from build123d import *

# Parameters (mm, degrees)
BASE_BODY_PROFILE_R   = 6.5
BASE_BODY_DEPTH       = 36
POCKET_32X20_SKETCH_W = 32
POCKET_32X20_SKETCH_H = 24
POCKET_32X20_DEPTH    = 110.840793879
LUG_ROUNDED_TOP_DEPTH = 14
LUG_BORE_34_REACH     = 128.4
LUG_BORE_SKETCH_R     = 17
BOSS_10MM_DEPTH       = 10
BOSS_BORE_SKETCH_R    = 12
BOSS_BORE_24_DEPTH    = 123.036879672


with BuildPart() as part:
    # Base Body Profile → Base Body (new, symmetric)
    with BuildSketch(Plane.XY):
        with BuildLine():
            Line((0, -12), (0, 0))
            Line((0, 0), (0, 55))
            Line((0, 55), (-14, 55))
            Line((-14, 55), (-14, 30))
            Line((-14, 30), (-28, 30))
            ThreePointArc((-28, 30), (-33.656854249, 27.656854249), (-36, 22))
            Line((-36, 22), (-36, 12))
            Line((-36, 12), (-94, 12))
            Line((-94, 12), (-94, 0))
            Line((-94, 0), (-88, 0))
            Line((-88, 0), (-88, -12))
            ThreePointArc((-88, -12), (-76, -24), (-64, -12))
            Line((-64, -12), (0, -12))
        make_face()
        with Locations((-76, -12)):
            Circle(BASE_BODY_PROFILE_R, mode=Mode.SUBTRACT)
    extrude(amount=BASE_BODY_DEPTH, both=True)

    # Pocket 32x20 Sketch → Pocket 32x20 (cut, through all)
    with BuildSketch(Plane.ZY.offset(88)):
        with Locations((0, -12)):
            Rectangle(POCKET_32X20_SKETCH_W, POCKET_32X20_SKETCH_H)
    extrude(amount=-POCKET_32X20_DEPTH, mode=Mode.SUBTRACT)

    # Lug Rounded Top Sketch → Lug Rounded Top (add)
    with BuildSketch(Plane(origin=(0, 0, 0), x_dir=(0, 0, -1), z_dir=(1, 0, 0))):
        with BuildLine():
            Line((-36, 55), (36, 55))
            ThreePointArc((36, 55), (0, 91), (-36, 55))
        make_face()
    extrude(amount=-LUG_ROUNDED_TOP_DEPTH)

    # Lug Bore Sketch → Lug Bore Ø34 (cut, up to next)
    with BuildSketch(Plane.ZY.offset(14), mode=Mode.PRIVATE) as lug_bore_34_sk1:
        with Locations(Location((0, 55, 0), (0, 0, 270))):
            Circle(LUG_BORE_SKETCH_R)
    lug_bore_34_tool1 = extrude(lug_bore_34_sk1.sketch, amount=-LUG_BORE_34_REACH, mode=Mode.PRIVATE) & part.part
    add(lug_bore_34_tool1.solids().sort_by_distance((-14, 55, 0))[0], mode=Mode.SUBTRACT)

    # Boss Profile 44x30 → Boss 10mm (add)
    with BuildSketch(Plane(origin=(0, 12, 0), x_dir=(1, 0, 0), z_dir=(0, 1, 0))):
        with BuildLine():
            Line((-66, 22), (-36, 22))
            Line((-36, 22), (-36, -22))
            Line((-36, -22), (-66, -22))
            ThreePointArc((-66, -22), (-88, 0), (-66, 22))
        make_face()
    extrude(amount=BOSS_10MM_DEPTH)

    # Boss Bore Sketch → Boss Bore Ø24 (cut, through all)
    with BuildSketch(Plane(origin=(0, 22, 0), x_dir=(1, 0, 0), z_dir=(0, 1, 0))):
        with Locations(Location((-66, 0, 0), (0, 0, 180))):
            Circle(BOSS_BORE_SKETCH_R)
    extrude(amount=-BOSS_BORE_24_DEPTH, mode=Mode.SUBTRACT)


solid = part.part
Geometry: final body of the model. Coordinates: model frame, mm. A direction names the side the tool comes from. Give positions to 0.01 mm unless a question says otherwise; leave off trailing zeros. Loops run counter-clockwise (first coordinate to the right, second up) from the corner with the lowest first, then second, coordinate; pieces in that order, holes last. Notation, with made-up numbers: (55, -28) -> (75, -28) arc R21 ccw to (75, 10) -> close; hole circle Ø9 at (41, 53). An arc over 180 degrees is marked (long way). Put each result on its own line as item: value.
1. Cut plane C-C (x = -76). Return the cut outline in (y, z).
Taken from the geometry:
outline: (-24, -36) -> (-18.5, -36) -> (-18.5, -16) -> (-24, -16) -> close; (-24, 16) -> (-18.5, 16) -> (-18.5, 36) -> (-24, 36) -> close; (-5.5, -36) -> (12, -36) -> (12, -19.6) -> (22, -19.6) -> (22, -6.63) -> (0, -6.63) -> (0, -16) -> (-5.5, -16) -> close; (-5.5, 16) -> (0, 16) -> (0, 6.63) -> (22, 6.63) -> (22, 19.6) -> (12, 19.6) -> (12, 36) -> (-5.5, 36) -> close
2. Cut plane A-A (z = 0). Return the cut outline in (x, y), plus the area to 3 significant figures.
Taken from the geometry:
outline: (-94, 0) -> (-78, 0) -> (-78, 22) -> (-88, 22) -> (-88, 12) -> (-94, 12) -> close; (-54, 0) -> (0, 0) -> (0, 38) -> (-14, 38) -> (-14, 30) -> (-28, 30) arc R8 ccw to (-36, 22) -> (-54, 22) -> close; (-14, 72) -> (0, 72) -> (0, 91) -> (-14, 91) -> close
area: 2,130 mm2
3. Ray query, line 1 along Y through (x, z) = (-76, 27.25); line 2 along Z through (x, y) = (-3.75, 55); line 3 along Y through (x, z) = (-52.5, 26). Return the intervals inside material, ascending. Write a range as [from, to].
Taken from the geometry:
line 1: y = [-24, -18.5], [-5.5, 12]
line 2: z = [-36, -17], [17, 36]
line 3: y = [-12, 12]
4. Cut plane B-B (x = -9). Return the cut outline in (y, z), plus the area to 3 significant figures.
Taken from the geometry:
outline: (-12, -36) -> (55, -36) arc R36 ccw to (55, 36) -> (-12, 36) -> (-12, 16) -> (0, 16) -> (0, -16) -> (-12, -16) -> close; hole circle Ø34 at (55, 0)
area: 5,570 mm2
5. Set-up query: faces 4 (the flat face through (-32, -12, 26)), 5 (the cylindrical face through (-88, 17, 0)), 6 (the flat face through (-36, 17, 29)), 7 (the flat face through (-88, -6, 26)), 8 (the flat face through (-51, 17, -22)). Return all of +Z, -Z, +X, -X, +Y, -Y with unobstructed straight access to the full face (end or side cutting, diameter ignored); none if empty.
Taken from the geometry:
face 4: +Z, -Z, +X, -Y
face 5: -X, +Y
face 6: +Z, -X, +Y
face 7: +Z, -Z, -X, -Y
face 8: -Z, -X, +Y
6. Pin query (flat end, axial travel): P1, Ø11, axis at x = -19, z = -3, coming from the +Y side; P2, Ø4, axis at y = -5.5, z = -19.5, coming from the +X side; P3, Ø3, axis at x = -16.5, z = -7, coming from the +Y side; P4, Ø6, axis at x = -19, z = -24, coming from the -Y side. Return the tip coordinate at first contact, or that it passes through.
Taken from the geometry:
P1: stops at y = 90.99
P2: stops at x = 0
P3: stops at y = 30
P4: stops at y = -12
7. Cut plane D-D (y = 10.5). Return the cut outline in (x, z).
Taken from the geometry:
outline: (-94, -36) -> (0, -36) -> (0, 36) -> (-94, 36) -> close; hole circle Ø24 at (-66, 0)
8. Pull-direction query (Y, two-part tool) for faces 1 (the cylindrical face through (-76, -24, -26)), 2 (the cylindrical face through (-70, -14.5, -26.1)), 3 (the flat face through (-94, 6, 1)); classes: released by +Y, released by -Y, zero draft, split by the parting line, or undercut.
Taken from the geometry:
face 1: released by -Y
face 2: undercut
face 3: zero draft
